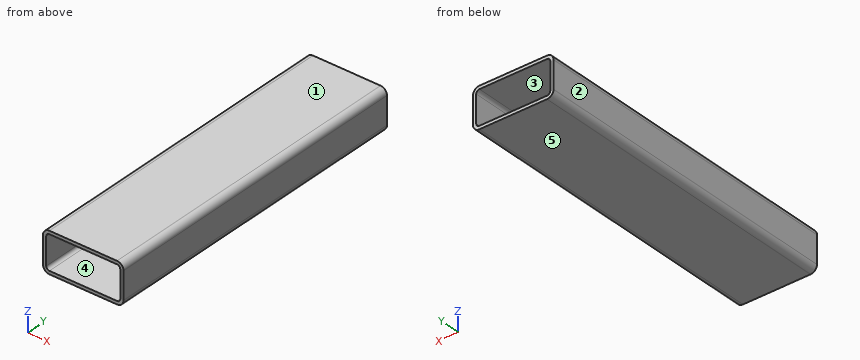
```python
from build123d import *

# Parameters (mm, degrees)
GB_T_6728_2002_RECTANGULAR_HOLLOW_SECTIO_DEPTH = 800


with BuildPart() as part:
    # Sketch12 → GB/T 6728-2002 rectangular hollow section 200X100X8(2) (new body)
    with BuildSketch(Plane.ZX):
        with BuildLine():
            Line((-34, -100), (34, -100))
            ThreePointArc((34, -100), (45.313708499, -95.313708499), (50, -84))
            Line((50, -84), (50, 84))
            ThreePointArc((50, 84), (45.313708499, 95.313708499), (34, 100))
            Line((34, 100), (-34, 100))
            ThreePointArc((-34, 100), (-45.313708499, 95.313708499), (-50, 84))
            Line((-50, 84), (-50, -84))
            ThreePointArc((-50, -84), (-45.313708499, -95.313708499), (-34, -100))
        make_face()
        with BuildLine():
            Line((-34, -92), (34, -92))
            ThreePointArc((34, -92), (39.656854249, -89.656854249), (42, -84))
            Line((42, -84), (42, 84))
            ThreePointArc((42, 84), (39.656854249, 89.656854249), (34, 92))
            Line((34, 92), (-34, 92))
            ThreePointArc((-34, 92), (-39.656854249, 89.656854249), (-42, 84))
            Line((-42, 84), (-42, -84))
            ThreePointArc((-42, -84), (-39.656854249, -89.656854249), (-34, -92))
        make_face(mode=Mode.SUBTRACT)
    extrude(amount=GB_T_6728_2002_RECTANGULAR_HOLLOW_SECTIO_DEPTH)


solid = part.part
```
Source: CAD feature listing. Evaluate the final solid. Frame: model axes, mm. Face numbers are marked on the shaded views. A direction names the side the tool comes from. Coordinates: 2 decimals unless noted, no trailing zeros. Order: outer loops, then holes, each group sorted by start corner. A loop starts at its lowest first (then second) coordinate and runs counter-clockwise, first axis right, second up. Notation, with made-up numbers: M 87,25.5 L 115,25.5 A24 ccw 115,38.5 Z; hole C -19,12 d10. An arc over 180 degrees is marked long. Write each question's results on one line, items separated by ' | '. Start each with the question number.
1) Contact query for a flat-ended pin moving along its axis: pin 1 Ø6 at (y, z) = (595.5, -39.5) entering from -X. Output: stop coordinate, or through.
2) Draft query along X for the marked faces 1, 2 and 3. Return one class per face: released by +X, released by -X, zero draft, split by the parting line, or undercut.
3) Section query A-A (x = -54.5). Return the cut outline in (y, z), plus the area to 3 significant figures.
4) Section query B-B (z = 17). Return the cut outline in (x, y).
5) Line query: line 1 (X direction, y = 714, z = 29.5); line 2 (Z direction, x = 31.5, y = 710); line 3 (X direction, y = 713, z = -40.5). Output: solid intervals per line, ascending. Write a range as from..to.
6) Section query C-C (y = 446). Return the cut outline in (x, z), plus the area to 3 significant figures.
7) Access query for the marked faces 4 and 5. Directions: +Z, -Z, +X, -X, +Y, -Y. A direction counts if a zero-diameter tool reaches every point of the face in a straight line with its end or side. Return the directions, or none.
Answers:
1) pin 1: stops at x = -99.8
2) face 1: zero draft | face 2: released by -X | face 3: undercut
3) outline: M 0,-50 L 800,-50 L 800,-42 L 0,-42 Z; M 0,42 L 800,42 L 800,50 L 0,50 Z | area: 12,800 mm^2
4) outline: M -100,0 L -92,0 L -92,800 L -100,800 Z; M 92,0 L 100,0 L 100,800 L 92,800 Z
5) line 1: x = -100..-92, 92..100 | line 2: z = -50..-42, 42..50 | line 3: x = -98.62..-88.66, 88.66..98.62
6) outline: M -100,-34 A16 ccw -84,-50 L 84,-50 A16 ccw 100,-34 L 100,34 A16 ccw 84,50 L -84,50 A16 ccw -100,34 Z; hole M -92,-34 A8 ccw -84,-42 L 84,-42 A8 ccw 92,-34 L 92,34 A8 ccw 84,42 L -84,42 A8 ccw -92,34 Z | area: 4,380 mm^2
7) face 4: +Y, -Y | face 5: -Z, +X, -X, +Y, -Y
